Source: CAD feature listing. Evaluate the final solid. Frame: model axes, mm. A direction names the side the tool comes from. Give positions to 0.01 mm unless a question says otherwise; leave off trailing zeros. Order: outer loops, then holes, each group sorted by start corner. A loop starts at its lowest first (then second) coordinate and runs counter-clockwise, first axis right, second up. Notation, with made-up numbers: M -21,40 L 27,40 A18 cw 27,55 Z; hole C -18.5,-34.5 d4. An arc over 180 degrees is marked long. Answer as a JSON object with one key per item and string values. Group by question number.
1. Section query C-C (z = -13). Output: boundary loops of the cut face in (x, y).
2. Section query A-A (y = 12). Output: boundary loops of the cut face in (x, z), plus the area to 3 significant figures.
3. Pin query (flat end, axial travel): P1, Ø12, axis at y = 83.5, z = -2.5, coming from the -X side; P2, Ø13, axis at x = 113, y = 26, coming from the -Z side; P3, Ø3, axis at x = 134, y = 73, coming from the -Z side; P4, Ø4, axis at x = 159, y = 3, coming from the -Z side. Return the tip coordinate at first contact, or that it passes through.
4. Pull-direction query (Y, two-part tool) for faces 1 (the flat face through (39, 0, 6)), 2 (the flat face through (190, 83, -5)), 3 (the cylindrical face through (110.615, 72.751, 6.93)); classes: +Y half, -Y half, draft (parallel to the pull), parting line (faces both ways), or undercut.
5. Section query B-B (x = 20). Output: boundary loops of the cut face in (y, z).
6. Set-up query: faces 4 (the cylindrical face through (108.381, 24.085, 0.986)), 5 (the flat face through (175, 37, 4)), 6 (the cylindrical face through (133.615, 3.751, 6.93)). Return all of +Z, -Z, +X, -X, +Y, -Y with unobstructed straight access to the full face (end or side cutting, diameter ignored); none if empty.
7. Section query D-D (y = 72). Count the separate pieces of the cut face and the enclosed holes in it, plus the area to 3 significant figures.
8. Material intervals for L1, parallel to Y at x = 136, z = 4.75; L2, parallel to Y at x = 136, z = 1.1; L3, parallel to Y at x = 20, z = 6.75, sorted ascending. Write a range as [from, to].
from build123d import *

# Parameters (mm, degrees)
BASE_PLATE_SKETCH_W       = 85
BASE_PLATE_SKETCH_H       = 75
BASE_PLATE_85X75_DEPTH    = 12
PLATE_EXTENSION_DEPTH     = 12
NOTCH_FILLET_R6_A_R       = 6
NOTCH_FILLET_R6_B_R       = 6
END_FLANGE_SKETCH_W       = 30
END_FLANGE_SKETCH_H       = 105
END_FLANGE_DEPTH          = 5
SIDE_TAB_1_SKETCH_W       = 15
SIDE_TAB_1_SKETCH_H       = 24
SIDE_TAB_1_DEPTH          = 15
SIDE_TAB_2_SKETCH_W       = 15
SIDE_TAB_2_SKETCH_H       = 24
SIDE_TAB_2_DEPTH          = 15
COUNTERBORE_GRID_SKETCH_R = 5
COUNTERBORES_12X_10_DEPTH = 2
HOLE_GRID_SKETCH_R        = 2.5
HOLE_GRID_12X_5_DEPTH     = 10
MOUNTING_HOLES_SKETCH_R   = 4
MOUNTING_HOLES_2X_8_DEPTH = 15


with BuildPart() as part:
    # Base Plate Sketch → Base Plate 85x75 (new body)
    with BuildSketch(Plane.XY):
        with Locations((42.5, 37.5)):
            Rectangle(BASE_PLATE_SKETCH_W, BASE_PLATE_SKETCH_H)
    extrude(amount=BASE_PLATE_85X75_DEPTH)

    # Plate Extension Sketch → Plate Extension (add)
    with BuildSketch(Plane.XY.offset(12)):
        Polygon((85, 75), (85, 37.5), (175, 37.5), (175, 90), (85, 90), align=None)
        Polygon((175, 37.5), (85, 37.5), (85, 0), (85, -15), (175, -15), align=None)
    extrude(amount=-PLATE_EXTENSION_DEPTH)

    # Notch Fillet R6 A
    notch_fillet_r6_a_edges = [part.edges().sort_by_distance(p)[0] for p in [
        (85, 75, 6),
    ]]
    fillet(notch_fillet_r6_a_edges, radius=NOTCH_FILLET_R6_A_R)

    # Notch Fillet R6 B
    notch_fillet_r6_b_edges = [part.edges().sort_by_distance(p)[0] for p in [
        (85, 0, 6),
    ]]
    fillet(notch_fillet_r6_b_edges, radius=NOTCH_FILLET_R6_B_R)

    # End Flange Sketch → End Flange (add)
    with BuildSketch(Plane.XY.offset(12)):
        with Locations((190, 37.5)):
            Rectangle(END_FLANGE_SKETCH_W, END_FLANGE_SKETCH_H)
    extrude(amount=-END_FLANGE_DEPTH)

    # Side Tab 1 Sketch → Side Tab 1 (add)
    with BuildSketch(Plane(origin=(0, 90, 0), x_dir=(1, 0, 0), z_dir=(0, 1, 0))):
        with Locations((197.5, 5)):
            Rectangle(SIDE_TAB_1_SKETCH_W, SIDE_TAB_1_SKETCH_H)
    extrude(amount=-SIDE_TAB_1_DEPTH)

    # Side Tab 2 Sketch → Side Tab 2 (add)
    with BuildSketch(Plane.XZ.offset(15)):
        with Locations((197.5, -5)):
            Rectangle(SIDE_TAB_2_SKETCH_W, SIDE_TAB_2_SKETCH_H)
    extrude(amount=-SIDE_TAB_2_DEPTH)

    # Counterbore Grid Sketch → Counterbores 12xØ10 (cut)
    with BuildSketch(Plane(origin=(0, 0, 0), x_dir=(-1, 0, 0), z_dir=(0, 0, -1))):
        with Locations((-159, 72)):
            Circle(COUNTERBORE_GRID_SKETCH_R)
        with Locations((-136, 72)):
            Circle(COUNTERBORE_GRID_SKETCH_R)
        with Locations((-113, 72)):
            Circle(COUNTERBORE_GRID_SKETCH_R)
        with Locations((-113, 49)):
            Circle(COUNTERBORE_GRID_SKETCH_R)
        with Locations((-136, 49)):
            Circle(COUNTERBORE_GRID_SKETCH_R)
        with Locations((-159, 49)):
            Circle(COUNTERBORE_GRID_SKETCH_R)
        with Locations((-159, 26)):
            Circle(COUNTERBORE_GRID_SKETCH_R)
        with Locations((-136, 26)):
            Circle(COUNTERBORE_GRID_SKETCH_R)
        with Locations((-113, 26)):
            Circle(COUNTERBORE_GRID_SKETCH_R)
        with Locations((-113, 3)):
            Circle(COUNTERBORE_GRID_SKETCH_R)
        with Locations((-136, 3)):
            Circle(COUNTERBORE_GRID_SKETCH_R)
        with Locations((-159, 3)):
            Circle(COUNTERBORE_GRID_SKETCH_R)
    extrude(amount=-COUNTERBORES_12X_10_DEPTH, mode=Mode.SUBTRACT)

    # Hole Grid Sketch → Hole Grid 12xØ5 (cut)
    with BuildSketch(Plane(origin=(0, 0, 2), x_dir=(-1, 0, 0), z_dir=(0, 0, -1))):
        with Locations((-159, 72)):
            Circle(HOLE_GRID_SKETCH_R)
        with Locations((-136, 72)):
            Circle(HOLE_GRID_SKETCH_R)
        with Locations((-113, 72)):
            Circle(HOLE_GRID_SKETCH_R)
        with Locations((-113, 49)):
            Circle(HOLE_GRID_SKETCH_R)
        with Locations((-136, 49)):
            Circle(HOLE_GRID_SKETCH_R)
        with Locations((-159, 49)):
            Circle(HOLE_GRID_SKETCH_R)
        with Locations((-159, 26)):
            Circle(HOLE_GRID_SKETCH_R)
        with Locations((-136, 26)):
            Circle(HOLE_GRID_SKETCH_R)
        with Locations((-113, 26)):
            Circle(HOLE_GRID_SKETCH_R)
        with Locations((-159, 3)):
            Circle(HOLE_GRID_SKETCH_R)
        with Locations((-136, 3)):
            Circle(HOLE_GRID_SKETCH_R)
        with Locations((-113, 3)):
            Circle(HOLE_GRID_SKETCH_R)
    extrude(amount=-HOLE_GRID_12X_5_DEPTH, mode=Mode.SUBTRACT)

    # Mounting Holes Sketch → Mounting Holes 2xØ8 (cut)
    with BuildSketch(Plane(origin=(0, 0, 0), x_dir=(-1, 0, 0), z_dir=(0, 0, -1))):
        with Locations((-20, 63)):
            Circle(MOUNTING_HOLES_SKETCH_R)
        with Locations((-20, 12)):
            Circle(MOUNTING_HOLES_SKETCH_R)
    extrude(amount=-MOUNTING_HOLES_2X_8_DEPTH, mode=Mode.SUBTRACT)


solid = part.part
Answer sheet:
{
 "1": {"outline": "M 190,-15 L 205,-15 L 205,0 L 190,0 Z; M 190,75 L 205,75 L 205,90 L 190,90 Z"},
 "2": {"outline": "M 0,0 L 16,0 L 16,12 L 0,12 Z; M 24,0 L 175,0 L 175,7 L 205,7 L 205,12 L 24,12 Z", "area": "2,150 mm^2"},
 "3": {"P1": "x = 84.22", "P2": "z = 0", "P3": "z = 2", "P4": "through"},
 "4": {"face 1": "-Y half", "face 2": "draft", "face 3": "undercut"},
 "5": {"outline": "M 0,0 L 8,0 L 8,12 L 0,12 Z; M 16,0 L 59,0 L 59,12 L 16,12 Z; M 67,0 L 75,0 L 75,12 L 67,12 Z"},
 "6": {"face 4": "-Z", "face 5": "-Z, +Y, -Y", "face 6": "+Z, -Z"},
 "7": {"separate pieces": "4", "enclosed holes": "0", "area": "2,040 mm^2"},
 "8": {"L1": "[-15, 0.5], [5.5, 23.5], [28.5, 46.5], [51.5, 69.5], [74.5, 90]", "L2": "[-15, -2], [8, 21], [31, 44], [54, 67], [77, 90]", "L3": "[0, 8], [16, 59], [67, 75]"}
}
